```python
from build123d import *

# Parameters (mm, degrees)
SKETCH_1_W          = 6.5
SKETCH_1_H          = 8
SKETCH_2_R          = 4
EXTRUDE_1_DEPTH     = 40
CUT_EXTRUDE_1_DEPTH = 4
CHAMFER_1_SIZE      = 0.65
CHAMFER_2_SIZE      = 0.767


with BuildPart() as part:
    # 草图1 → 旋转1 (revolve)
    with BuildSketch(Plane(origin=(0, 0, 0), x_dir=(1, 0, 0), z_dir=(0, 1, 0))):
        with Locations((3.25, -4)):
            Rectangle(SKETCH_1_W, SKETCH_1_H)
    revolve(axis=Axis((0, 0, 0), (0, 0, 1)))

    # 草图2 → 凸台-拉伸1 (add)
    with BuildSketch(Plane(origin=(0, 0, 0), x_dir=(-1, 0, 0), z_dir=(0, 0, -1))):
        Circle(SKETCH_2_R)
    extrude(amount=EXTRUDE_1_DEPTH)

    # 草图3 → 切除-拉伸1 (cut)
    with BuildSketch(Plane.XY.offset(8)):
        Polygon((3, 1.732050808), (0, 3.464101615), (-3, 1.732050808), (-3, -1.732050808), (0, -3.464101615), (3, -1.732050808), align=None)
    extrude(amount=-CUT_EXTRUDE_1_DEPTH, mode=Mode.SUBTRACT)

    # 草图4 → 切除-旋转1 (revolve, cut)
    with BuildSketch(Plane.XZ, mode=Mode.PRIVATE) as cut_revolve_1_sk:
        Polygon((3, 4), (0, 4), (0, 2.267949192), align=None)
    revolve(cut_revolve_1_sk.sketch.rotate(Axis((0, 0, 4), (0, 0, -1)), 90), axis=Axis((0, 0, 4), (0, 0, -1)), mode=Mode.SUBTRACT)

    # 倒角1
    chamfer_1_edges = [part.edges().sort_by_distance(p)[0] for p in [
        (-6.5, 0, 8),
    ]]
    chamfer(chamfer_1_edges, length=CHAMFER_1_SIZE)

    # 倒角2
    chamfer_2_edges = [part.edges().sort_by_distance(p)[0] for p in [
        (4, 0, -40),
    ]]
    chamfer(chamfer_2_edges, length=CHAMFER_2_SIZE)


solid = part.part
```
Verification items for the finished model (mm, model axes). A direction names the side the tool comes from. Round coordinates to 2 decimals unless told otherwise and drop trailing zeros. Write each loop counter-clockwise with the first axis right and the second up, starting at its lowest first coordinate (ties: lowest second). Pieces come first, ordered by that corner, then holes.
1. Gauge pin test, flat ends, axial feed: P1, Ø1, axis at x = -3.5, y = 3, coming from the -Z side; P2, Ø1.5, axis at x = -0.5, z = -31.5, coming from the -Y side; P3, Ø1.5, axis at y = 1, z = 1.5, coming from the -X side. Record the tip position at first contact, or that the pin passes through.
2. Scan lines: L1, parallel to Z at x = 5, y = -1; L2, parallel to X at y = 2, z = -36; L3, parallel to Z at x = 0.25, y = 3. Record each from-to range of solid material in increasing order.
3. Section check B-B on z = 1.5. Enter the section's corners in (x, y), plus the area to 3 significant figures.
4. Section check A-A on z = -35.5. Enter the section's corners in (x, y), plus the area to 3 significant figures.
5. Access from +Z, -Z, +X, -X, +Y, -Y to the whole of each face (thin tool, end or side, straight path). Record for faces 5 (the flat face through (-3, 3, 0)), 6 (the flat face through (-1.5, 2.6, 6)), 7 (the cylindrical face through (-5.158, -3.955, 3.624)).
6. Draft check along X on faces 1 (the cylindrical face through (0.867, -3.905, -19.342)), 2 (the flat face through (-3, -3, 8)), 3 (the flat face through (-2.8, -1.6, 4)), 4 (the flat face through (-3, 0, 6)). Enter one of: +X half, -X half, draft (parallel to the pull), parting line (faces both ways), or undercut.
Answer:
1. P1: stops at z = 0
1. P2: stops at y = -4
1. P3: stops at x = -6.5
2. L1: z = 0 to 8
2. L2: x = -3.46 to 3.46
2. L3: z = -40 to 4
3. outline: circle Ø13 at (0, 0)
3. area: 133 mm2
4. outline: circle Ø8 at (0, 0)
4. area: 50.3 mm2
5. face 5: -Z
5. face 6: +Z
5. face 7: +Z, -Z
6. face 1: parting line
6. face 2: draft
6. face 3: undercut
6. face 4: undercut
